from build123d import *

# Parameters (mm, degrees)
SKETCH_1_W                = 100
SKETCH_1_H                = 55
EXTRUDE_1_DEPTH           = 25
SKETCH_2_W                = 48.2
SKETCH_2_H                = 4
CUT_EXTRUDE_1_DEPTH       = 107.682941467
HOLE_WIZARD_M5_1_D        = 4.2
HOLE_WIZARD_M5_1_DEPTH    = 12.4
HOLE_WIZARD_M5_1_TIP      = 1.2618073
CHAMFER_1_SIZE            = 1
HOLE_WIZARD_0_D           = 6.6
HOLE_WIZARD_0_DEPTH       = 40
HOLE_WIZARD_0_CBORE_D     = 11
HOLE_WIZARD_0_CBORE_DEPTH = 6.8
HOLE_WIZARD_0_TIP         = 1.982840043
HOLE_WIZARD_M5_2_D        = 4.2
HOLE_WIZARD_M5_2_DEPTH    = 12.4
HOLE_WIZARD_M5_2_TIP      = 1.2618073
MM_1_D                    = 5
MM_1_DEPTH                = 12.4
MM_1_TIP                  = 1.502151548


with BuildPart() as part:
    # 草图1 → 凸台-拉伸1 (new body)
    with BuildSketch(Plane(origin=(0, 0, 0), x_dir=(1, 0, 0), z_dir=(0, 1, 0))):
        Rectangle(SKETCH_1_W, SKETCH_1_H)
    extrude(amount=EXTRUDE_1_DEPTH)

    # 草图2 → 切除-拉伸1 (cut, through all)
    with BuildSketch(Plane(origin=(50, 0, 0), x_dir=(0, 0, -1), z_dir=(1, 0, 0))):
        Rectangle(SKETCH_2_W, SKETCH_2_H)
    extrude(amount=-CUT_EXTRUDE_1_DEPTH, mode=Mode.SUBTRACT)

    # M5 螺纹孔1
    with Locations(Plane.XY.offset(27.5)):
        with Locations((42.5, 20), (42.5, 5), (-42.5, 20), (-42.5, 5)):
            Hole(HOLE_WIZARD_M5_1_D / 2, depth=HOLE_WIZARD_M5_1_DEPTH)
            with Locations((0, 0, -(HOLE_WIZARD_M5_1_DEPTH + HOLE_WIZARD_M5_1_TIP / 2))):  # 118° drill point
                Cone(0, HOLE_WIZARD_M5_1_D / 2, HOLE_WIZARD_M5_1_TIP, mode=Mode.SUBTRACT)

    # 倒角1
    chamfer_1_edges = [part.edges().sort_by_distance(p)[0] for p in [
        (50, 12.5, 27.5),
        (-50, 12.5, 27.5),
        (-50, 12.5, -27.5),
        (50, 12.5, -27.5),
    ]]
    chamfer(chamfer_1_edges, length=CHAMFER_1_SIZE)

    # 打孔尺寸(%根据)内六角圆柱头螺钉的类型0
    with Locations(Plane(origin=(0, 25, 0), x_dir=(1, 0, 0), z_dir=(0, 1, 0))):
        with Locations((-17.499999996, 17.499999996), (17.500000004, 17.499999996), (-17.499999996, -17.500000004), (17.500000004, -17.500000004)):
            CounterBoreHole(HOLE_WIZARD_0_D / 2, HOLE_WIZARD_0_CBORE_D / 2, HOLE_WIZARD_0_CBORE_DEPTH, depth=HOLE_WIZARD_0_DEPTH)
            with Locations((0, 0, -(HOLE_WIZARD_0_DEPTH + HOLE_WIZARD_0_TIP / 2))):  # 118° drill point
                Cone(0, HOLE_WIZARD_0_D / 2, HOLE_WIZARD_0_TIP, mode=Mode.SUBTRACT)

    # M5 螺纹孔2
    with Locations(Plane(origin=(0, 25, 0), x_dir=(1, 0, 0), z_dir=(0, 1, 0))):
        with Locations((-35, 17.5), (-35, -17.5), (35, 17.5), (35, -17.5), (0, 17.5), (0, -17.5)):
            Hole(HOLE_WIZARD_M5_2_D / 2, depth=HOLE_WIZARD_M5_2_DEPTH)
            with Locations((0, 0, -(HOLE_WIZARD_M5_2_DEPTH + HOLE_WIZARD_M5_2_TIP / 2))):  # 118° drill point
                Cone(0, HOLE_WIZARD_M5_2_D / 2, HOLE_WIZARD_M5_2_TIP, mode=Mode.SUBTRACT)

    # 大小mm 暗销孔1
    with Locations(Plane(origin=(0, 25, 0), x_dir=(1, 0, 0), z_dir=(0, 1, 0))):
        with Locations((-30, 0), (30, 0)):
            Hole(MM_1_D / 2, depth=MM_1_DEPTH)
            with Locations((0, 0, -(MM_1_DEPTH + MM_1_TIP / 2))):  # 118° drill point
                Cone(0, MM_1_D / 2, MM_1_TIP, mode=Mode.SUBTRACT)


solid = part.part
Here's how the part is built. I have some questions about the finished solid (model axes, mm). A direction names the side the tool comes from. Coordinates: 2 decimals unless noted, no trailing zeros. Write each loop counter-clockwise with the first axis right and the second up, starting at its lowest first coordinate (ties: lowest second). Pieces come first, ordered by that corner, then holes.
Item 1: I want a section at B-B on x = 6. Write out the boundary of the cut face in (y, z).
Item 2: Will these pins go through, and if not, where does the flat tip stop? pin 1 (5 mm diameter, centred on x = -35, z = 17.5, fed in from +Y); pin 2 (3 mm diameter, centred on x = -30, z = 0, fed in from -Y); pin 3 (3.5 mm diameter, centred on x = 42.5, y = 5, fed in from +Z); pin 4 (4 mm diameter, centred on x = -17.5, z = 17.5, fed in from +Y).
Item 3: If I drill on line 1 (Z direction, x = 0, y = 16.5); line 2 (X direction, y = 20, z = 24.5); line 3 (Z direction, x = 17.5, y = 21.25), over which ranges is the centre line in solid material (lowest first)?
Item 4: I want a section at C-C on z = -22. Write out the boundary of the cut face in (x, y), and give its area (3 significant figures).
Item 5: If we mould it in two halves opening along Y, with no side actions, what happens to faces 5 (the conical face through (42.85, 5.11, 14.06)), 6 (the cylindrical face through (-1.13, 18.71, -19.27)), 7 (the flat face through (-1, 25, 0))? For each: +Y half, -Y half, draft (parallel to the pull), parting line (faces both ways), or undercut.
Item 6: On a 3-axis mill with a long thin cutter (end or side, diameter ignored), from which of +Z, -Z, +X, -X, +Y, -Y can I reach the whole of each face in a straight line? I mean faces 1 (the cylindrical face through (42.773, 7.082, 21.213)), 2 (the flat face through (-1, 12, -27.5)), 3 (the flat face through (1, 1, 24.1)), 4 (the flat face through (20, 18.2, 20)). Say none if no direction works.
Item 7: I want a section at A-A on y = 16.5. Count the separate pieces of the cut face and the enclosed holes in it, and give its area (3 significant figures).
Findings below:
1. outline: (0, -27.5) - (25, -27.5) - (25, 27.5) - (0, 27.5) - (0, 24.1) - (2, 24.1) - (2, -24.1) - (0, -24.1) - close
2. pin 1: stops at y = 25
2. pin 2: stops at y = 2
2. pin 3: stops at z = 14.89
2. pin 4: passes through
3. line 1: z = -27.5 to -19.6, -15.4 to 15.4, 19.6 to 27.5
3. line 2: x = -50 to -44.6, -40.4 to 40.4, 44.6 to 50
3. line 3: z = -27.5 to -23, -12 to 12, 23 to 27.5
4. outline: (-50, 2) - (50, 2) - (50, 25) - (20.66, 25) - (20.66, 18.2) - (14.34, 18.2) - (14.34, 25) - (-14.34, 25) - (-14.34, 18.2) - (-20.66, 18.2) - (-20.66, 25) - (-50, 25) - close
4. area: 2,210 mm2
5. face 5: undercut
5. face 6: draft
5. face 7: +Y half
6. face 1: +Z
6. face 2: -Z, +X, -X, +Y, -Y
6. face 3: +X, -X, -Y
6. face 4: +Y
7. separate pieces: 1
7. enclosed holes: 12
7. area: 5,240 mm2
